Source: three-view drawing plus pictorial views. Frame: mm from the lowest corner of the part. Give positions to 0.01 mm unless a question says otherwise; leave off trailing zeros. Loops run counter-clockwise (first coordinate to the right, second up) from the corner with the lowest first, then second, coordinate; pieces in that order, holes last. Notation, with made-up numbers: (58.5, -6.5) -> (86.5, -6.5) arc R16 cw to (86.5, 22.5) -> close; hole circle Ø8 at (65.25, 63.25). An arc over 180 degrees is marked (long way). Put each result on its own line as item: value.
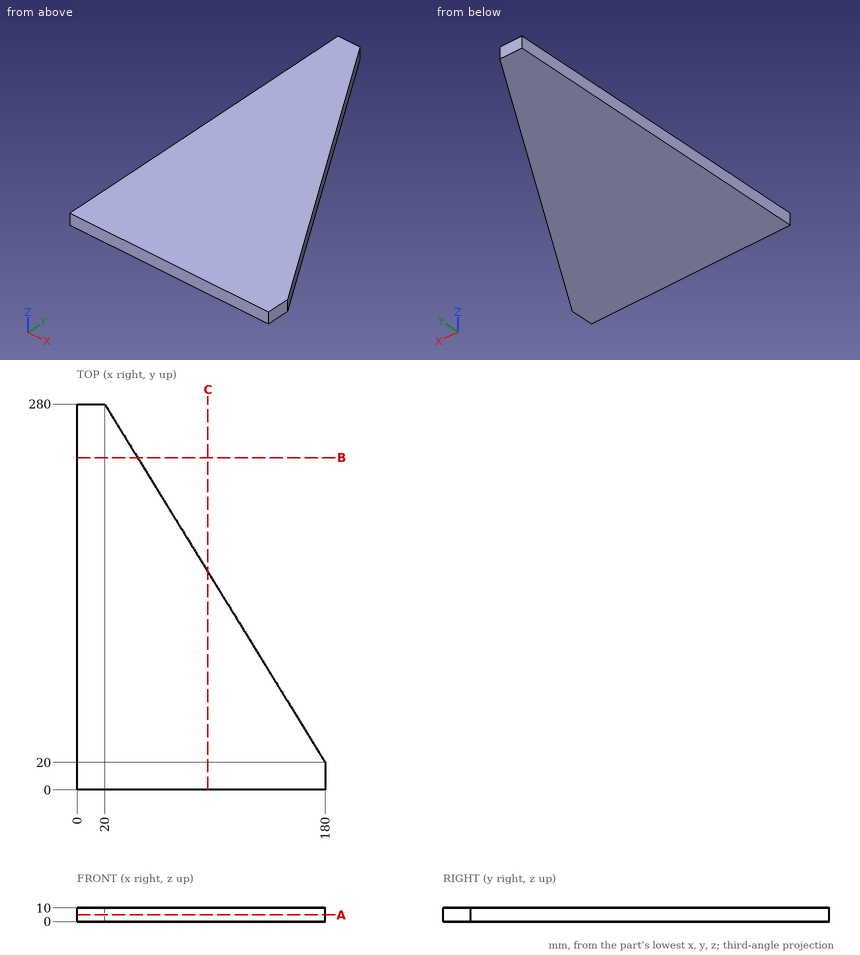
(1) Section C-C on x = 95. Return loops of the section in (y, z) (3 decimals).
Calculated:
outline: (0, 0) -> (158.125, 0) -> (158.125, 10) -> (0, 10) -> close
(2) First-contact query: P1, Ø3, axis at x = 83, z = 6, coming from the -Y side; P2, Ø3, axis at x = 106.5, z = 6.5, coming from the +Y side (3 decimals). Flat tips, straight axial feed; report the tip coordinate or a pass-through.
Calculated:
P1: stops at y = 0
P2: stops at y = 141.875
(3) Section A-A on z = 5. Return loops of the section in (x, y), then the cut area to 3 significant figures.
Calculated:
outline: (0, 0) -> (180, 0) -> (180, 20) -> (20, 280) -> (0, 280) -> close
area: 29,600 mm²
(4) Section B-B on y = 241. Return loops of the section in (x, z).
Calculated:
outline: (0, 0) -> (44, 0) -> (44, 10) -> (0, 10) -> close
(5) Line query: probe 1 along X at (y, z) = (53, 4.75); probe 2 along X at (y, z) = (74.5, 0.75); probe 3 along Y at (x, z) = (42.5, 4.25). Output: solid intervals per line, ascending. Write a range as from..to.
Calculated:
probe 1: x = 0..159.69
probe 2: x = 0..146.46
probe 3: y = 0..243.44
